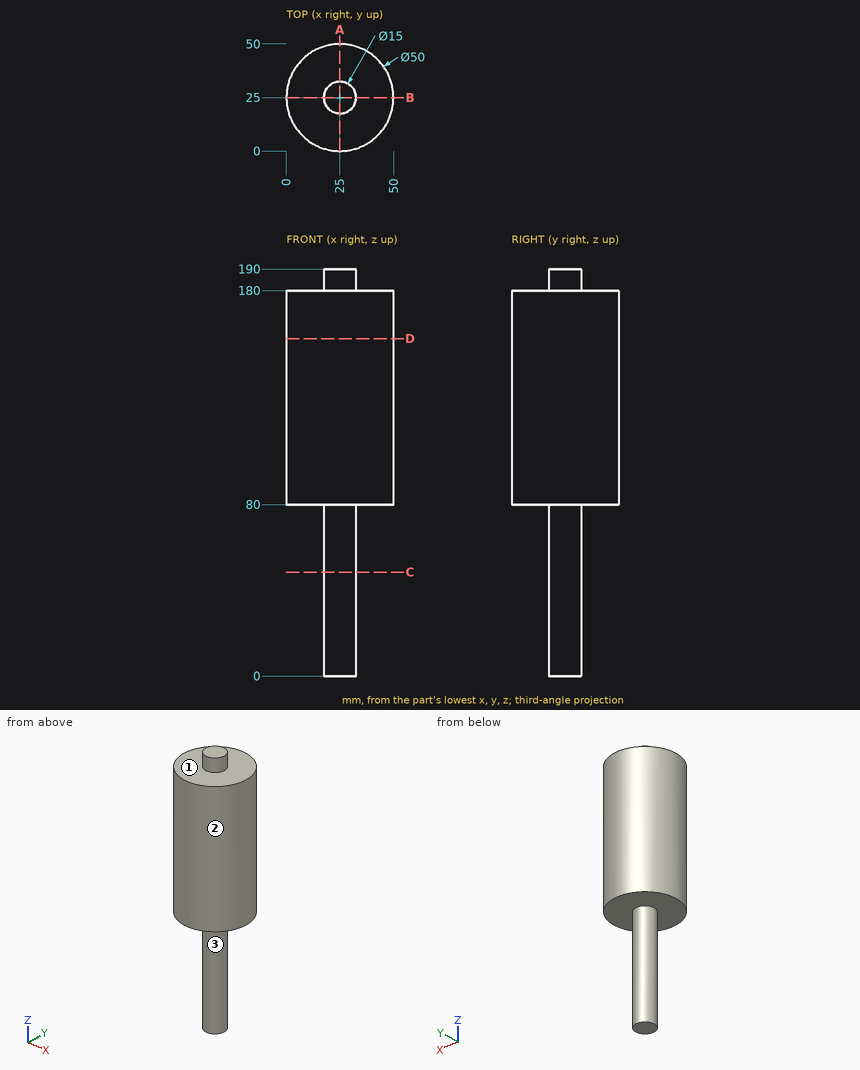
Can you work these out from the drawing? Everything is in mm from the part's minimum corner. A direction names the side the tool comes from. Round coordinates to 2 decimals unless told otherwise and drop trailing zeros. Loops run counter-clockwise (first coordinate to the right, second up) from the corner with the lowest first, then second, coordinate; pieces in that order, holes last. Notation, with made-up numbers: (-21, 48.5) - (-5, 48.5) arc R31 ccw to (-5, 75.5) - close; hole circle Ø6 at (67, 1). An arc over 180 degrees is marked (long way). Answer in a Markdown table with one row per item. Add a question column.
Q1. For pin 1 Ø2 at (x, y) = (7.5, 13) entering from +Z; pin 2 Ø10 at (x, z) = (41.5, 168) entering from -Y; pin 3 Ø8 at (x, z) = (22, 163) entering from -Y, each with a flat end and sliding along its axis, tell me the tip position at first contact or that it passes through.
Q2. Which directions (+Z, -Z, +X, -X, +Y, -Y) give clear straight access to the entire face, cutting with the end or side of a thin tool? Please do the marked faces 1, 2 and 3.
Q3. I want a section at A-A on x = 25. List the corners of the cut face in (y, z) for me, and give its area (3 significant figures).
Q4. I need wall thicknesses on L1, parallel to Z at x = 13.5, y = 14.5; L2, parallel to Y at x = 21, z = 16; L3, parallel to X at y = 12.5, z = 97.5. Which ranges of each line are inside material? Lowest first, please.
Q5. I want a section at D-D on z = 157.5. List the corners of the cut face in (x, y) for me, and give its area (3 significant figures).
Q6. I want a section at C-C on z = 48.5. List the corners of the cut face in (x, y) for me.
A:
| question | item | result |
|---|---|---|
| 1 | pin 1 | z = 180 |
| 1 | pin 2 | y = 2.8 |
| 1 | pin 3 | y = 0 |
| 2 | face 1 | +Z |
| 2 | face 2 | +Z, -Z |
| 2 | face 3 | -Z |
| 3 | outline | (0, 80) - (17.5, 80) - (17.5, 0) - (32.5, 0) - (32.5, 80) - (50, 80) - (50, 180) - (32.5, 180) - (32.5, 190) - (17.5, 190) - (17.5, 180) - (0, 180) - close |
| 3 | area | 6,350 mm^2 |
| 4 | L1 | 80 to 180 |
| 4 | L2 | 18.66 to 31.34 |
| 4 | L3 | 3.35 to 46.65 |
| 5 | outline | circle Ø50 at (25, 25) |
| 5 | area | 1,960 mm^2 |
| 6 | outline | circle Ø15 at (25, 25) |
